Can you work these out from the model? Positions are in its coordinate system, mm. Round coordinates to 2 decimals unless told otherwise and drop trailing zeros. Loops run counter-clockwise (first coordinate to the right, second up) from the corner with the lowest first, then second, coordinate; pieces in that order, holes last. Notation, with made-up numbers: (-10.5, 1) - (1.5, 1) arc R15 cw to (1.5, 14) - close; hole circle Ø3 at (73, 18.25). An arc over 180 degrees is marked (long way). Answer as CSV lines item,"result".
```python
from build123d import *

# Parameters (mm, degrees)
EXTRUDE_1_DEPTH = 10


with BuildPart() as part:
    # 草图2 → 拉伸-薄壁1 (new, symmetric)
    with BuildSketch(Plane.XY):
        with BuildLine():
            Line((-69.067097429, -255.055208246), (-100.763322879, -13.205809086))
            ThreePointArc((-100.763322879, -13.205809085), (-6.616945736, 101.40935193), (101.624999966, 2.2e-08))
            Line((101.624999966, 2.2e-08), (101.624999966, -634.999999978))
            ThreePointArc((101.624999966, -634.999999978), (-4.66638799, -736.517808507), (-101.196460274, -625.677068041))
            Line((-101.196460274, -625.677068041), (-68.719202326, -273.150248716))
            ThreePointArc((-68.719202326, -273.150248716), (-68.390081735, -264.093056497), (-69.067097429, -255.055208246))
        make_face()
        with BuildLine():
            Line((-59.151887309, -253.755743635), (-90.848112759, -11.906344475))
            ThreePointArc((-90.848112759, -11.906344475), (-5.965831768, 91.430571914), (91.624999966, 2.2e-08))
            Line((91.624999966, 2.2e-08), (91.624999966, -634.999999978))
            ThreePointArc((91.624999966, -634.999999978), (-4.207210823, -726.528356253), (-91.238629008, -626.594453717))
            Line((-91.238629008, -626.594453717), (-58.76137106, -274.067634393))
            ThreePointArc((-58.76137106, -274.067634393), (-58.391929417, -263.900832101), (-59.151887309, -253.755743635))
        make_face(mode=Mode.SUBTRACT)
    extrude(amount=EXTRUDE_1_DEPTH, both=True)


solid = part.part
```
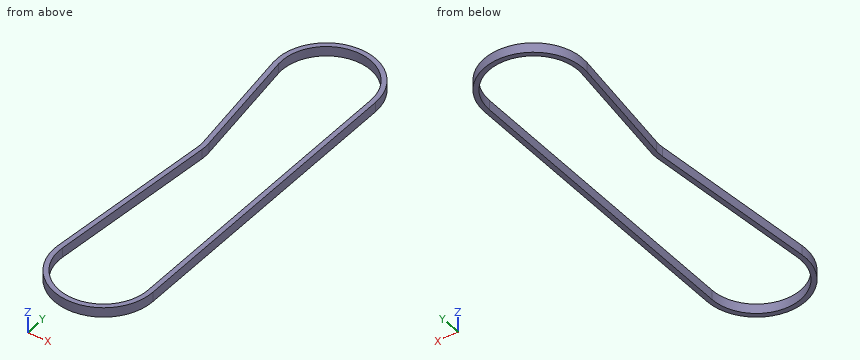
Q1. Imagine slicing it at A-A (x = 0). Write out the boundary of the cut face in (y, z) (3 decimals).
Checks:
outline,"(-736.625, -10) - (-726.625, -10) - (-726.625, 10) - (-736.625, 10) - close; (91.625, -10) - (101.625, -10) - (101.625, 10) - (91.625, 10) - close"
Q2. If I drill on line 1 along X through (y, z) = (-471.5, 7) (3 decimals); line 2 along X through (y, z) = (-339, -3.25) (3 decimals); line 3 along Y through (x, z) = (59, -5.75), over which ranges is the centre line in solid material (lowest first)? Write a range as [from, to].
Checks:
line 1,"[-86.993, -76.95], [91.625, 101.625]"
line 2,"[-74.786, -64.743], [91.625, 101.625]"
line 3,"[-717.74, -705.1], [70.1, 82.74]"
Q3. I'm going to push flat-ended pins straight in: pin 1 Ø10 at (y, z) = (-384.5, 3.5) entering from -X; pin 2 Ø4 at (x, z) = (-55.5, 8) entering from -Y; pin 3 Ø5 at (y, z) = (-3.5, 6.5) entering from -X. Where does each tip first touch, or does it pass through?
Checks:
pin 1,"x = -79.44"
pin 2,"y = -721.4"
pin 3,"x = -101.62"
Q4. Imagine slicing it at B-B (y = -230). Write out the boundary of the cut face in (x, z) (3 decimals), then the cut area to 3 significant figures.
Checks:
outline,"(-72.351, -10) - (-62.265, -10) - (-62.265, 10) - (-72.351, 10) - close; (91.625, -10) - (101.625, -10) - (101.625, 10) - (91.625, 10) - close"
area,"402 mm²"
Q5. Imagine slicing it at C-C (z = -3.5). Write out the boundary of the cut face in (x, y) (3 decimals).
Checks:
outline,"(-101.196, -625.677) arc R101.625 ccw (long way) to (101.625, -635) - (101.625, 0) arc R101.625 ccw (long way) to (-100.763, -13.206) - (-69.067, -255.055) arc R81.625 cw to (-68.719, -273.15) - close; hole (-91.239, -626.594) arc R91.625 ccw (long way) to (91.625, -635) - (91.625, 0) arc R91.625 ccw (long way) to (-90.848, -11.906) - (-59.152, -253.756) arc R91.625 cw to (-58.761, -274.068) - close"
